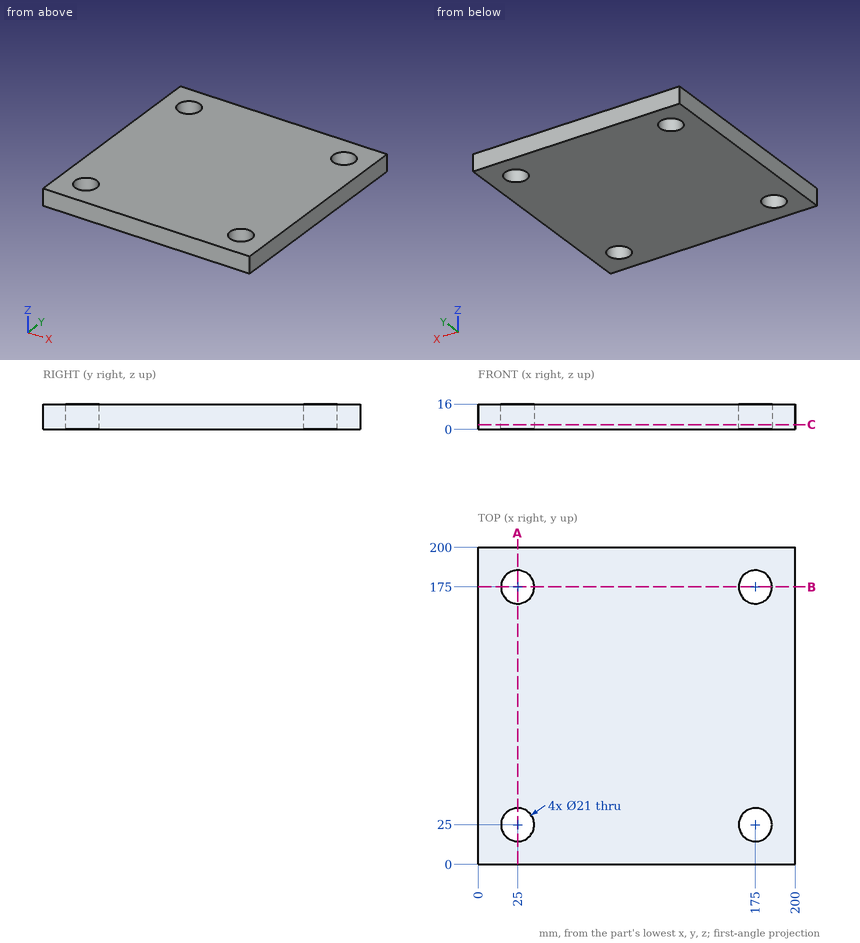
Input: dimensioned drawing with shaded views. Units: mm. Origin: part minimum x, y, z. Coordinates: 2 decimals unless noted, no trailing zeros. Order: outer loops, then holes, each group sorted by start corner. A loop starts at its lowest first (then second) coordinate and runs counter-clockwise, first axis right, second up. Notation, with made-up numbers: (31.5, 3) - (78.5, 3) arc R29 cw to (78.5, 35) - close; hole circle Ø1 at (4, 47). An arc over 180 degrees is marked (long way). One line per item, written item: value.
1) Cut plane A-A on x = 25. Output: boundary loops of the cut face in (y, z).
Computed values:
outline: (0, 0) - (14.5, 0) - (14.5, 16) - (0, 16) - close; (35.5, 0) - (164.5, 0) - (164.5, 16) - (35.5, 16) - close; (185.5, 0) - (200, 0) - (200, 16) - (185.5, 16) - close
2) Ray query, line 1 (Y direction, x = 175, z = 7.25); line 2 (X direction, y = 166.5, z = 2.25); line 3 (Y direction, x = 183, z = 5.5). Return the intervals inside material, ascending. Write a range as [from, to].
Computed values:
line 1: y = [0, 14.5], [35.5, 164.5], [185.5, 200]
line 2: x = [0, 18.84], [31.16, 168.84], [181.16, 200]
line 3: y = [0, 18.2], [31.8, 168.2], [181.8, 200]
3) Contact query for flat-ended pins moving along their axis: pin 1 (8 mm diameter, centred on y = 98, z = 3.5, fed in from -X); pin 2 (17 mm diameter, centred on x = 25, y = 25, fed in from -Z). Output: stop coordinate, or through.
Computed values:
pin 1: stops at x = 0
pin 2: passes through
4) Cut plane C-C on z = 3. Output: boundary loops of the cut face in (x, y), plus the area to 3 significant figures.
Computed values:
outline: (0, 0) - (200, 0) - (200, 200) - (0, 200) - close; hole circle Ø21 at (25, 25); hole circle Ø21 at (25, 175); hole circle Ø21 at (175, 25); hole circle Ø21 at (175, 175)
area: 38,600 mm^2
